Can you work these out from the model? Positions are in its coordinate system, mm. A direction names the side the tool comes from. Coordinates: 2 decimals unless noted, no trailing zeros. Order: outer loops, then holes, each group sorted by start corner. A loop starts at its lowest first (then second) coordinate and runs counter-clockwise, first axis right, second up.
```python
from build123d import *

# Parameters (mm, degrees)
EXTRUDE_1_DEPTH            = 15
SKETCH_2_R                 = 27.5
EXTRUDE_2_DEPTH            = 396
HOLE_WIZARD_1_D            = 9
HOLE_WIZARD_1_CBORE_D      = 15
HOLE_WIZARD_1_CBORE_DEPTH  = 6
CHAMFER_1_SIZE             = 1.5
CHAMFER_1_OF_MIRROR_1_SIZE = 1.5
SKETCH_5_W                 = 2
SKETCH_5_H                 = 100
CUT_EXTRUDE_1_DEPTH        = 424.878815229


with BuildPart() as part:
    # 草图1 → 凸台-拉伸1 (new body)
    with BuildSketch(Plane(origin=(0, 0, 0), x_dir=(0, 0, -1), z_dir=(1, 0, 0))):
        with BuildLine():
            Line((-62.5, 24), (62.5, 24))
            Line((62.5, 24), (62.5, -24))
            Line((62.5, -24), (-62.5, -24))
            ThreePointArc((-62.5, -24), (-86.5, 0), (-62.5, 24))
        make_face()
    extrude_1 = extrude(amount=EXTRUDE_1_DEPTH)

    # 草图2 → 凸台-拉伸2 (add)
    with BuildSketch(Plane.ZY):
        with Locations(Location((62.5, 0, 0), (0, 0, 240.777129706))):
            Circle(SKETCH_2_R)
    extrude(amount=EXTRUDE_2_DEPTH)

    # 打孔尺寸(%根据)内六角花形圆柱头螺钉1 (through all)
    with Locations(Plane(origin=(15, 0, 0), x_dir=(0, 0, -1), z_dir=(1, 0, 0))):
        with Locations((17.5, 0), (47.5, 0)):
            hole_wizard_1 = CounterBoreHole(HOLE_WIZARD_1_D / 2, HOLE_WIZARD_1_CBORE_D / 2, HOLE_WIZARD_1_CBORE_DEPTH)

    # 倒角1
    chamfer_1_edges = [part.edges().sort_by_distance(p)[0] for p in [
        (15, 0, 86.5),
        (15, -24, 0),
        (15, 0, -62.5),
        (15, 24, 0),
    ]]
    chamfer(chamfer_1_edges, length=CHAMFER_1_SIZE)

    # 镜向1: 凸台-拉伸1, 打孔尺寸(%根据)内六角花形圆柱头螺钉1 across plane
    add(extrude_1.mirror(Plane.ZY.offset(198)))
    add(hole_wizard_1.mirror(Plane.ZY.offset(198)), mode=Mode.SUBTRACT)

    # 倒角1 of 镜向1
    chamfer_1_of_mirror_1_edges = [part.edges().sort_by_distance(p)[0] for p in [
        (-411, 0, 86.5),
        (-411, -24, 0),
        (-411, 0, -62.5),
        (-411, 24, 0),
    ]]
    chamfer(chamfer_1_of_mirror_1_edges, length=CHAMFER_1_OF_MIRROR_1_SIZE)

    # 草图5 → 切除-拉伸1 (cut, through all)
    with BuildSketch(Plane(origin=(0, 24, 0), x_dir=(1, 0, 0), z_dir=(0, 1, 0))):
        with Locations((-397, 12.5)):
            Rectangle(SKETCH_5_W, SKETCH_5_H)
        with Locations((1, 12.5)):
            Rectangle(SKETCH_5_W, SKETCH_5_H)
    extrude(amount=-CUT_EXTRUDE_1_DEPTH, mode=Mode.SUBTRACT)


solid = part.part
```
1. Imagine slicing it at B-B on z = 19. Please give me the cut outline in (x, y).
Completed:
outline: (-411, -22.5) - (-409.5, -24) - (-398, -24) - (-398, 24) - (-409.5, 24) - (-411, 22.5) - close; (2, -24) - (13.5, -24) - (15, -22.5) - (15, 22.5) - (13.5, 24) - (2, 24) - close
2. Please list where these lines run through material, in increasing order: probe 1 along Z at (x, y) = (-402, 0); probe 2 along Z at (x, y) = (-408, 0); probe 3 along X at (y, z) = (11, 36).
Completed:
probe 1: z = -62.5 to -52, -43 to -22, -13 to 86.5
probe 2: z = -62.5 to -55, -40 to -25, -10 to 86.5
probe 3: x = -411 to -398, 2 to 15
3. Imagine slicing it at C-C on y = 0. Give the number of separate pieces and of enclosed holes in the cut face, then the cut area to 3 significant figures.
Completed:
separate pieces: 5
enclosed holes: 0
area: 25,200 mm2
4. Imagine slicing it at D-D on x = -319. Please give me the cut outline in (y, z), then the cut area to 3 significant figures.
Completed:
outline: circle Ø55 at (0, 62.5)
area: 2,380 mm2
5. Thinking about a two-plate mould opening in Z: for faces 4 (the flat face through (-411, 0, 11)), 5 (the flat face through (-405, 0.1, -22.4)), 6 (the cylindrical face through (-402.656, -0.528, 86.494)), which applies, pulls with the +Z half, pulls with the -Z half, needs draft (parallel to the pull), parting line crosses it, or undercut?
Completed:
face 4: needs draft
face 5: undercut
face 6: pulls with the +Z half
6. I'm going to push flat-ended pins straight in: pin 1 (1.6 mm diameter, centred on x = -397, y = 8, fed in from -Z); pin 2 (11 mm diameter, centred on x = 4, z = -19.5, fed in from -Y); pin 3 (12 mm diameter, centred on x = -322, z = 70.5, fed in from +Y). Where does each tip first touch, or does it pass through?
Completed:
pin 1: stops at z = 37.5
pin 2: stops at y = -24
pin 3: stops at y = 27.43
7. Imagine slicing it at A-A on z = -17.5. Please give me the cut outline in (x, y).
Completed:
outline: (-411, -22.5) - (-409.5, -24) - (-398, -24) - (-398, -4.5) - (-405, -4.5) - (-405, -7.5) - (-411, -7.5) - close; (-411, 7.5) - (-405, 7.5) - (-405, 4.5) - (-398, 4.5) - (-398, 24) - (-409.5, 24) - (-411, 22.5) - close; (2, -24) - (13.5, -24) - (15, -22.5) - (15, -7.5) - (9, -7.5) - (9, -4.5) - (2, -4.5) - close; (2, 4.5) - (9, 4.5) - (9, 7.5) - (15, 7.5) - (15, 22.5) - (13.5, 24) - (2, 24) - close
8. On a 3-axis mill with a long thin cutter (end or side, diameter ignored), from which of +Z, -Z, +X, -X, +Y, -Y can I reach the whole of each face in a straight line? I mean faces 1 (the flat face through (0, -20, 41)), 2 (the cylindrical face through (-195.228, -10.187, 88.044)), 3 (the flat face through (-405, -5, -47)). Say none if no direction works.
Completed:
face 1: -Z, -Y
face 2: none
face 3: -X
